Could you check a few things on this model? Use its own coordinates, in mm. Face numbers are marked on the shaded views. A direction names the side the tool comes from. Give positions to 0.01 mm unless a question says otherwise; leave off trailing zeros. Write each loop counter-clockwise with the first axis right and the second up, starting at its lowest first coordinate (ties: lowest second). Pieces come first, ordered by that corner, then holes. Notation, with made-up numbers: (72, 0) -> (122, 0) arc R11 cw to (122, 4) -> close; hole circle Ø11 at (36.25, 49). An arc over 180 degrees is marked (long way). One line per question, with ' | ' between items.
from build123d import *

# Parameters (mm, degrees)
CUT_EXTRUDE1_DEPTH = 47.368092477


with BuildPart() as part:
    # Sketch1 → Revolve1 (revolve)
    with BuildSketch(Plane.XY, mode=Mode.PRIVATE) as revolve1_sk:
        Polygon((-10, 0), (-10, -30), (-25, -30), (-25, -25), (-18, -25), (-18, -5), (-25, -5), (-25, 0), align=None)
    revolve(revolve1_sk.sketch.rotate(Axis((0, 76.758624558, 0), (0, -1, 0)), 270), axis=Axis((0, 76.758624558, 0), (0, -1, 0)))

    # Sketch2 → Cut-Extrude1 (cut, through all)
    with BuildSketch(Plane(origin=(0, 0, 0), x_dir=(1, 0, 0), z_dir=(0, 1, 0))):
        with BuildLine():
            Line((-2.5, 12.682458366), (-2.5, 9.682458366))
            ThreePointArc((-2.5, 9.682458366), (0, 10), (2.5, 9.682458366))
            Line((2.5, 9.682458366), (2.5, 12.682458366))
            Line((2.5, 12.682458366), (-2.5, 12.682458366))
        make_face()
    extrude(amount=-CUT_EXTRUDE1_DEPTH, mode=Mode.SUBTRACT)


solid = part.part
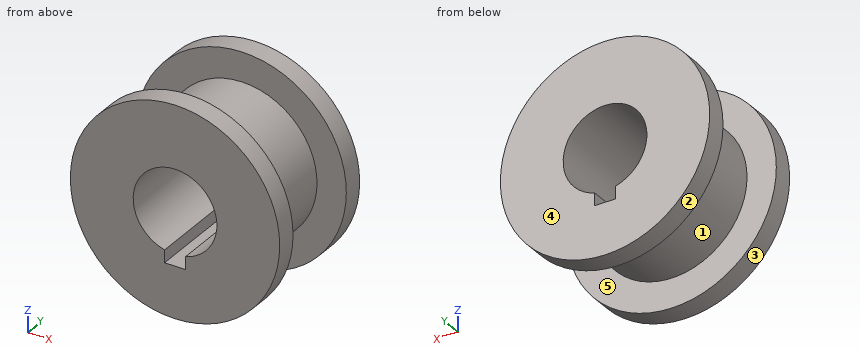
Q1. Imagine slicing it at C-C on y = -22.5. Please give me the cut outline in (x, z), and give its area (3 significant figures).
Answer below:
outline: circle Ø36 at (0, 0); hole (-2.5, -12.68) -> (2.5, -12.68) -> (2.5, -9.68) arc R10 ccw (long way) to (-2.5, -9.68) -> close | area: 690 mm^2
Q2. If we mould it in two halves opening along Y, with no side actions, what happens to the marked faces 3, 4 and 5? For each: +Y half, -Y half, draft (parallel to the pull), parting line (faces both ways), or undercut.
Answer below:
face 3: draft | face 4: +Y half | face 5: undercut
Q3. Imagine slicing it at D-D on y = -26. Please give me the cut outline in (x, z), and give its area (3 significant figures).
Answer below:
outline: circle Ø50 at (0, 0); hole (-2.5, -12.68) -> (2.5, -12.68) -> (2.5, -9.68) arc R10 ccw (long way) to (-2.5, -9.68) -> close | area: 1,640 mm^2
Q4. Imagine slicing it at B-B on x = 0. Please give me the cut outline in (y, z).
Answer below:
outline: (-30, -25) -> (-25, -25) -> (-25, -18) -> (-5, -18) -> (-5, -25) -> (0, -25) -> (0, -12.68) -> (-30, -12.68) -> close; (-30, 10) -> (0, 10) -> (0, 25) -> (-5, 25) -> (-5, 18) -> (-25, 18) -> (-25, 25) -> (-30, 25) -> close
Q5. Imagine slicing it at A-A on z = 0. Please give me the cut outline in (x, y), and give its area (3 significant figures).
Answer below:
outline: (-25, -30) -> (-10, -30) -> (-10, 0) -> (-25, 0) -> (-25, -5) -> (-18, -5) -> (-18, -25) -> (-25, -25) -> close; (10, -30) -> (25, -30) -> (25, -25) -> (18, -25) -> (18, -5) -> (25, -5) -> (25, 0) -> (10, 0) -> close | area: 620 mm^2
Q6. If I drill on line 1 along X through (y, z) = (-22, 0); line 2 along Y through (x, z) = (20, -2); line 3 along X through (y, z) = (-26, 0), over which ranges is the centre line in solid material (lowest first)?
Answer below:
line 1: x = -18 to -10, 10 to 18 | line 2: y = -30 to -25, -5 to 0 | line 3: x = -25 to -10, 10 to 25
Q7. Will these pins go through, and if not, where does the flat tip stop? pin 1 (3.5 mm diameter, centred on y = -10, z = -11, fed in from +X); pin 2 (5.5 mm diameter, centred on x = 0.5, y = -18, fed in from +Z); pin 3 (8 mm diameter, centred on x = -13.5, y = -11.5, fed in from +Z); pin 4 (4 mm diameter, centred on x = 10.5, z = 12, fed in from +Y).
Answer below:
pin 1: stops at x = 15.44 | pin 2: stops at z = 18 | pin 3: stops at z = 15.29 | pin 4: stops at y = 0
Q8. On a 3-axis mill with a long thin cutter (end or side, diameter ignored), from which of +Z, -Z, +X, -X, +Y, -Y can I reach the whole of each face in a straight line? I mean the marked faces 1 and 2. Say none if no direction works.
Answer below:
face 1: none | face 2: +Y, -Y
